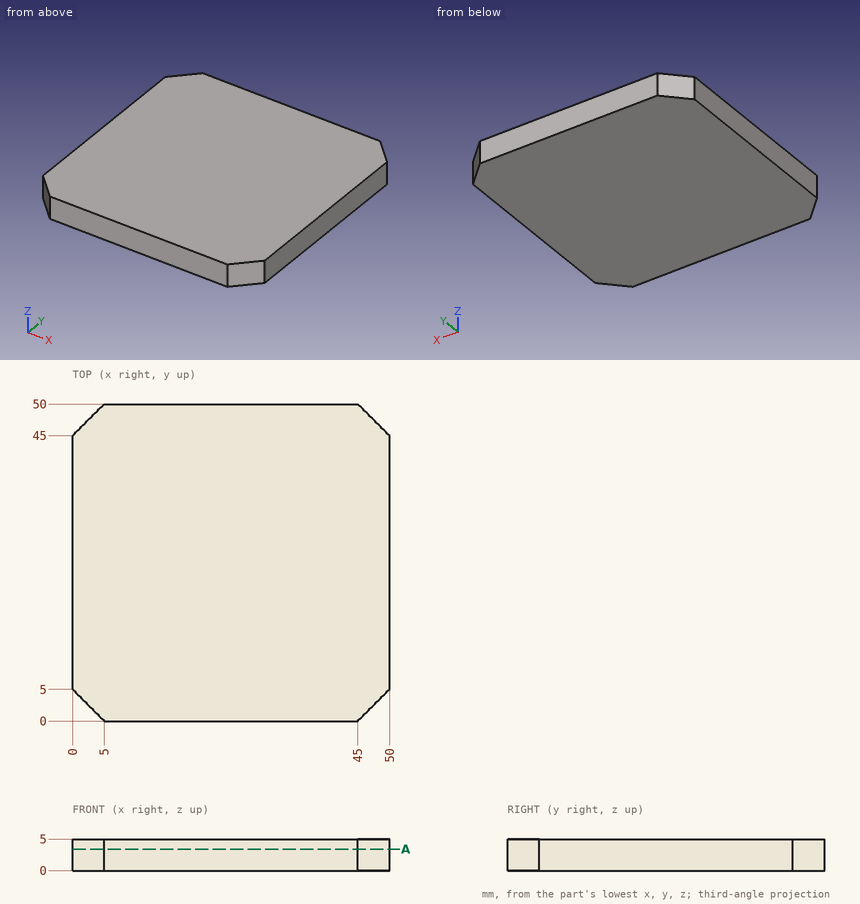
Geometry check sheet. Reference: drawing and pictorial views, mm from the part's lowest x, y, z. Coordinates: 2 decimals unless noted, no trailing zeros. Order: outer loops, then holes, each group sorted by start corner. A loop starts at its lowest first (then second) coordinate and runs counter-clockwise, first axis right, second up. Notation, with made-up numbers: (-33, 12) - (-15, 12) arc R15 ccw to (-15, 24) - close; hole circle Ø3 at (-24.5, 59.5). An arc over 180 degrees is marked (long way). One line per item, written item: value.
(1) Thickness scan on probe 1 along X at (y, z) = (46.5, 3.7); probe 2 along Y at (x, z) = (4, 3.15); probe 3 along X at (y, z) = (3, 0.7). Record the ranges inside material, lowest first. Write a range as from..to.
Data:
probe 1: x = 1.5..48.5
probe 2: y = 1..49
probe 3: x = 2..48
(2) Sectioned sample at A-A (z = 3.4). Enter the section's corners in (x, y), and give its area (3 significant figures).
Data:
outline: (0, 5) - (5, 0) - (45, 0) - (50, 5) - (50, 45) - (45, 50) - (5, 50) - (0, 45) - close
area: 2,450 mm^2
(3) Depth check by flat-ended pin: pin 1 Ø5 at (x, y) = (41.5, 42) entering from -Z. Enter the tip coordinate at first touch or a pass-through.
Data:
pin 1: stops at z = 0
